Model file for the job. Use its own axes, mm. A direction names the side the tool comes from. Give positions to 0.01 mm unless a question says otherwise; leave off trailing zeros. Loops run counter-clockwise (first coordinate to the right, second up) from the corner with the lowest first, then second, coordinate; pieces in that order, holes last. Notation, with made-up numbers: (-23, 18) -> (-19, 18) arc R28 cw to (-19, 43) -> close; hole circle Ø3 at (-10.5, 86.5). An arc over 180 degrees is marked (long way). Use CSV: the item, a comma, the result in double quotes. Start each with the question number.
(1) Drill centre lines: probe 1 along Y at (x, z) = (0.75, 4); probe 2 along Y at (x, z) = (-8.5, -0.75); probe 3 along X at (y, z) = (29.5, 0). Where is each one in solid material? Low to high.
(2) Cut at A-A on z = 0. Write the cut outline in (x, y), then the cut area to 3 significant figures.
(3) 3-axis set-ups, long thin cutter, end or side, ignore diameter. For faces 1 (the flat face through (-2, 47.2, 4)), 2 (the cylindrical face through (-9.76, 9.86, -2.17)): which of +Z, -Z, +X, -X, +Y, -Y reach the whole face in a straight line?
(4) Cut at B-B on x = 0. Write the cut outline in (y, z).
(5) Cut at D-D on x = -4.75. Write the cut outline in (y, z).
(6) Flat gauge pins, fed straight in: pin 1 (2 mm diameter, centred on x = 6, z = -6, fed in from +Y); pin 2 (12 mm diameter, centred on y = 63.5, z = 3.5, fed in from +X); pin 3 (5 mm diameter, centred on y = 43, z = 5.5, fed in from -X). Where does each tip first touch, or does it go through?
(7) Pull direction X, two halves, no side cores. Call faces 3 (the flat face through (-7.4, 20, -4.5)), 4 (the flat face through (0, 57, -2.8)), 5 (the cylindrical face through (-1.532, 61.99, 3.695)): pulls with the +X half, pulls with the -X half, needs draft (parallel to the pull), parting line crosses it, or undercut.
(8) Cut at C-C on y = 14. Write the cut outline in (x, z).
from build123d import *

# Parameters (mm, degrees)
SKETCH1_R           = 10
BOSS_EXTRUDE1_DEPTH = 20
SKETCH2_R           = 8.5
BOSS_EXTRUDE2_DEPTH = 27.2
SKETCH3_R           = 4
BOSS_EXTRUDE3_DEPTH = 30
CUT_EXTRUDE1_DEPTH  = 1.2


with BuildPart() as part:
    # Sketch1 → Boss-Extrude1 (new body)
    with BuildSketch(Plane(origin=(0, 0, 0), x_dir=(1, 0, 0), z_dir=(0, 1, 0))):
        with Locations(Location((0, 0, 0), (0, 0, 270))):
            Circle(SKETCH1_R)
    extrude(amount=BOSS_EXTRUDE1_DEPTH)

    # Sketch2 → Boss-Extrude2 (add)
    with BuildSketch(Plane(origin=(0, 20, 0), x_dir=(1, 0, 0), z_dir=(0, 1, 0))):
        with Locations(Location((0, 0, 0), (0, 0, 270))):
            Circle(SKETCH2_R)
    extrude(amount=BOSS_EXTRUDE2_DEPTH)

    # Sketch3 → Boss-Extrude3 (add)
    with BuildSketch(Plane(origin=(0, 47.2, 0), x_dir=(1, 0, 0), z_dir=(0, 1, 0))):
        with Locations(Location((0, 0, 0), (0, 0, 270))):
            Circle(SKETCH3_R)
    extrude(amount=BOSS_EXTRUDE3_DEPTH)

    # Sketch4 → Cut-Extrude1 (cut)
    with BuildSketch(Plane(origin=(0, 0, -4), x_dir=(-1, 0, 0), z_dir=(0, 0, -1))):
        with BuildLine():
            Line((-1, 50.2), (-1, 64.2))
            ThreePointArc((-1, 64.2), (0, 65.2), (1, 64.2))
            Line((1, 64.2), (1, 50.2))
            ThreePointArc((1, 50.2), (0, 49.2), (-1, 50.2))
        make_face()
    extrude(amount=-CUT_EXTRUDE1_DEPTH, mode=Mode.SUBTRACT)


solid = part.part
Check result:
1,probe 1,"0 to 47.2"
1,probe 2,"0 to 20"
1,probe 3,"-8.5 to 8.5"
2,outline,"(-10, 0) -> (10, 0) -> (10, 20) -> (8.5, 20) -> (8.5, 47.2) -> (4, 47.2) -> (4, 77.2) -> (-4, 77.2) -> (-4, 47.2) -> (-8.5, 47.2) -> (-8.5, 20) -> (-10, 20) -> close"
2,area,"1,100 mm²"
3,face 1,"+Y"
3,face 2,"+Y, -Y"
4,outline,"(0, -10) -> (20, -10) -> (20, -8.5) -> (47.2, -8.5) -> (47.2, -4) -> (49.2, -4) -> (49.2, -2.8) -> (65.2, -2.8) -> (65.2, -4) -> (77.2, -4) -> (77.2, 4) -> (47.2, 4) -> (47.2, 8.5) -> (20, 8.5) -> (20, 10) -> (0, 10) -> close"
5,outline,"(0, -8.8) -> (20, -8.8) -> (20, -7.05) -> (47.2, -7.05) -> (47.2, 7.05) -> (20, 7.05) -> (20, 8.8) -> (0, 8.8) -> close"
6,pin 1,"y = 47.2"
6,pin 2,"x = 4"
6,pin 3,"x = -7.95"
7,face 3,"needs draft"
7,face 4,"undercut"
7,face 5,"parting line crosses it"
8,outline,"circle Ø20 at (0, 0)"
